from build123d import *

# Parameters (mm, degrees)
SKETCH1_W                                           = 500
SKETCH1_H                                           = 24
BOSS_EXTRUDE1_DEPTH                                 = 400
SKETCH2_W                                           = 430
SKETCH2_H                                           = 8
CUT_EXTRUDE1_DEPTH                                  = 641.762046317
SKETCH3_W                                           = 544.957019416
SKETCH3_H                                           = 0.5
CUT_EXTRUDE2_DEPTH                                  = 641.762046317
SKETCH12_W                                          = 569.007892772
SKETCH12_H                                          = 39.328779912
CUT_EXTRUDE3_DEPTH                                  = 641.762046317
HOLE_WIZARD_HEX_SOCKET_SEMI_COUNTERSUNK_D           = 9
HOLE_WIZARD_HEX_SOCKET_SEMI_COUNTERSUNK_CSINK_D     = 17.6
HOLE_WIZARD_HEX_SOCKET_SEMI_COUNTERSUNK_CSINK_ANGLE = 90
SKETCH16_W                                          = 24
SKETCH16_H                                          = 60
SKETCH16_W_2                                        = 20
CUT_EXTRUDE4_DEPTH                                  = 2
FILLET1_R                                           = 5
HOLE_WIZARD_HEX_SOCKET_SEMI_COUNTER_2_D             = 9
HOLE_WIZARD_HEX_SOCKET_SEMI_COUNTER_2_CSINK_D       = 17.6
HOLE_WIZARD_HEX_SOCKET_SEMI_COUNTER_2_CSINK_ANGLE   = 90


with BuildPart() as part:
    # Sketch1 → Boss-Extrude1 (new body)
    with BuildSketch(Plane.XY):
        with Locations((250, 12)):
            Rectangle(SKETCH1_W, SKETCH1_H)
    extrude(amount=-BOSS_EXTRUDE1_DEPTH)

    # Sketch2 → Cut-Extrude1 (cut, through all)
    with BuildSketch(Plane.XY):
        with Locations((250, 12)):
            Rectangle(SKETCH2_W, SKETCH2_H)
    extrude(amount=-CUT_EXTRUDE1_DEPTH, mode=Mode.SUBTRACT)

    # Sketch3 → Cut-Extrude2 (cut, through all)
    with BuildSketch(Plane.XY):
        with Locations((250, 12)):
            Rectangle(SKETCH3_W, SKETCH3_H)
    extrude(amount=-CUT_EXTRUDE2_DEPTH, mode=Mode.SUBTRACT)


with BuildPart() as cut_extrude2_piece_1:
    # of the separate pieces the step leaves, piece 1, a body of its own (cut_extrude2_pieces)
    add(part.part.solids().sort_by_distance((0, 0, 0))[0])

    # Hole wizard_ hex socket semi-countersunk (through all)
    with Locations(Plane(origin=(0, 11.75, 0), x_dir=(1, 0, 0), z_dir=(0, 1, 0))):
        with Locations((20, 20), (480, 20), (20, 380), (480, 380)):
            CounterSinkHole(HOLE_WIZARD_HEX_SOCKET_SEMI_COUNTERSUNK_D / 2, HOLE_WIZARD_HEX_SOCKET_SEMI_COUNTERSUNK_CSINK_D / 2, counter_sink_angle=HOLE_WIZARD_HEX_SOCKET_SEMI_COUNTERSUNK_CSINK_ANGLE)

    # Sketch16 → Cut-Extrude4 (cut)
    with BuildSketch(Plane(origin=(0, 11.75, 0), x_dir=(1, 0, 0), z_dir=(0, 1, 0))):
        with Locations((12, 330)):
            Rectangle(SKETCH16_W, SKETCH16_H)
        with Locations((12, 70)):
            Rectangle(SKETCH16_W, SKETCH16_H)
        with Locations((10, 200)):
            Rectangle(SKETCH16_W_2, SKETCH16_H)
    extrude(amount=-CUT_EXTRUDE4_DEPTH, mode=Mode.SUBTRACT)

    # Fillet1
    fillet1_edges = [cut_extrude2_piece_1.edges().sort_by_distance(p)[0] for p in [
        (24, 10.75, -360),
        (24, 10.75, -300),
        (24, 10.75, -40),
        (24, 10.75, -100),
        (20, 10.75, -230),
        (20, 10.75, -170),
    ]]
    fillet(fillet1_edges, radius=FILLET1_R)

    # Hole wizard_ hex socket semi-counter 2 (through all)
    with Locations(Plane(origin=(0, 11.75, 0), x_dir=(1, 0, 0), z_dir=(0, 1, 0))):
        with Locations((20, 140), (20, 260), (480, 200)):
            CounterSinkHole(HOLE_WIZARD_HEX_SOCKET_SEMI_COUNTER_2_D / 2, HOLE_WIZARD_HEX_SOCKET_SEMI_COUNTER_2_CSINK_D / 2, counter_sink_angle=HOLE_WIZARD_HEX_SOCKET_SEMI_COUNTER_2_CSINK_ANGLE)


with BuildPart() as cut_extrude2_piece_2:
    # of the separate pieces the step leaves, piece 2, a body of its own (cut_extrude2_pieces)
    add(part.part.solids().sort_by_distance((0, 24, 0))[0])

    # Sketch12 → Cut-Extrude3 (cut, through all)
    with BuildSketch(Plane.XY):
        with Locations((265.175540793, 31.664389956)):
            Rectangle(SKETCH12_W, SKETCH12_H)
    extrude(amount=-CUT_EXTRUDE3_DEPTH, mode=Mode.SUBTRACT)


solid = cut_extrude2_piece_1.part
Can you work these out from the model? Positions are in its coordinate system, mm. A direction names the side the tool comes from. Coordinates: 2 decimals unless noted, no trailing zeros. Loops run counter-clockwise (first coordinate to the right, second up) from the corner with the lowest first, then second, coordinate; pieces in that order, holes last. Notation, with made-up numbers: M 77.25,57.25 L 102.25,57.25 A13 ccw 102.25,70.25 Z; hole C -10.75,72.25 d10. An arc over 180 degrees is marked long. Return JSON: item names as keys, results as strings. Group by question number.
Item 1: Thinking about a two-plate mould opening in X: for faces 1 (the flat face through (12, 9.75, -70)), 2 (the flat face through (247, 8, -197)), 3 (the flat face through (500, 6, -197)), which applies, released by +X, released by -X, zero draft, split by the parting line, or undercut?
Item 2: Imagine slicing it at A-A (z = -163). Please give me the cut outline in (x, y), and give its area (3 significant figures).
Item 3: Imagine slicing it at B-B (x = 453). Please give me the cut outline in (y, z), and give its area (3 significant figures).
Item 4: On a 3-axis mill with a long thin cutter (end or side, diameter ignored), from which of +Z, -Z, +X, -X, +Y, -Y can I reach the whole of each face in a straight line? I mean faces 4 (the flat face through (12, 9.75, -330)), 5 (the conical face through (475.65, 7.66, -18.2)). Say none if no direction works.
Item 5: Imagine slicing it at C-C (z = -71.5). Please give me the cut outline in (x, y), and give its area (3 significant figures).
Item 6: If I drill on L1, parallel to X at y = 5.75, z = -380; L2, parallel to Z at x = 480, y = 4.5; L3, parallel to Z at x = 20, y = 5.25, over which ranges is the centre line in solid material (lowest first)? Write a range as from..to.
Item 7: I'm going to push flat-ended pins straight in: pin 1 Ø1.6 at (y, z) = (11, -331.5) entering from -X; pin 2 Ø7 at (x, z) = (8, -316.5) entering from +Y; pin 3 Ø3 at (x, z) = (61.5, -97) entering from +Y. Where does each tip first touch, or does it pass through?
Verdict:
{
 "1": {"face 1": "zero draft", "face 2": "undercut", "face 3": "released by +X"},
 "2": {"outline": "M 0,0 L 500,0 L 500,11.75 L 465,11.75 L 465,8 L 35,8 L 35,11.75 L 0,11.75 Z", "area": "4,260 mm^2"},
 "3": {"outline": "M 0,-400 L 8,-400 L 8,0 L 0,0 Z", "area": "3,200 mm^2"},
 "4": {"face 4": "-X, +Y", "face 5": "+Y"},
 "5": {"outline": "M 0,0 L 500,0 L 500,11.75 L 465,11.75 L 465,8 L 35,8 L 35,11.75 L 24,11.75 L 24,9.75 L 0,9.75 Z", "area": "4,210 mm^2"},
 "6": {"L1": "x = 0..15.5, 24.5..475.5, 484.5..500", "L2": "z = -400..-384.5, -375.5..-204.5, -195.5..-24.5, -15.5..0", "L3": "z = -400..-384.5, -375.5..-264.5, -255.5..-144.5, -135.5..-24.5, -15.5..0"},
 "7": {"pin 1": "stops at x = 24", "pin 2": "stops at y = 9.75", "pin 3": "stops at y = 8"}
}
